The model under review builds one solid part; all positions refer to its coordinate system, in mm. Coordinates: 2 decimals unless noted, no trailing zeros. Loops run counter-clockwise (first coordinate to the right, second up) from the corner with the lowest first, then second, coordinate; pieces in that order, holes last. Notation, with made-up numbers: M -22,36 L -12,36 A27 cw -12,54 Z; hole C -32,69 d10. An arc over 180 degrees is marked long. One line per item, written item: value.
```python
from build123d import *

# Parameters (mm, degrees)
SKETCH1_W           = 39
SKETCH1_H           = 20
BOSS_EXTRUDE1_DEPTH = 620
CHAMFER1_SIZE       = 8


with BuildPart() as part:
    # Sketch1 → Boss-Extrude1 (new body)
    with BuildSketch(Plane.XY):
        with Locations((19.5, 10)):
            Rectangle(SKETCH1_W, SKETCH1_H)
    extrude(amount=BOSS_EXTRUDE1_DEPTH)

    # Chamfer1
    chamfer1_edges = [part.edges().sort_by_distance(p)[0] for p in [
        (0, 20, 310),
    ]]
    chamfer(chamfer1_edges, length=CHAMFER1_SIZE)


solid = part.part
```
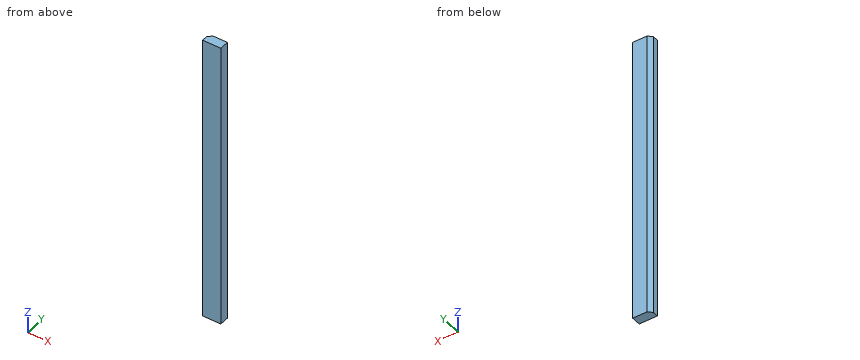
(1) Insertion check: pin 1 Ø1.5 at (x, z) = (7, 446.5) entering from +Y. The pin has a flat end and moves straight along its axis. Give the tip position at first contact, or say it passes through.
Checks:
pin 1: y = 19.75
(2) Add section B-B on y = 15.5. State the section outline as (x, z) points, then the cut area to 3 significant figures.
Checks:
outline: M 3.5,0 L 39,0 L 39,620 L 3.5,620 Z
area: 22,000 mm^2
(3) Add section A-A on z = 38. State the section outline as (x, y) points.
Checks:
outline: M 0,0 L 39,0 L 39,20 L 8,20 L 0,12 Z
(4) To check wall thickness, follow L1, parallel to X at y = 17.75, z = 205.5; L2, parallel to Y at x = 4, z = 310.5; L3, parallel to X at y = 16, z = 223.5. State the ranges of each line that lie inside material, in increasing order. Write a range as [from, to].
Checks:
L1: [5.75, 39]
L2: [0, 16]
L3: [4, 39]
